```python
from build123d import *

# Parameters (mm, degrees)
SKETCH1_W      = 310
SKETCH1_H      = 180
SKETCH1_R      = 8.5
SKETCH1_R_2    = 8
EXTRUDE1_DEPTH = 6


with BuildPart() as part:
    # Sketch1 → Extrude1 (new, symmetric)
    with BuildSketch(Plane(origin=(0, 0, 0), x_dir=(1, 0, 0), z_dir=(0, 1, 0))):
        Rectangle(SKETCH1_W, SKETCH1_H)
        with Locations(Location((125, -65, 0), (0, 0, 270))):
            Circle(SKETCH1_R, mode=Mode.SUBTRACT)
        with Locations(Location((-125, -65, 0), (0, 0, 270))):
            Circle(SKETCH1_R_2, mode=Mode.SUBTRACT)
        with Locations(Location((-125, 65, 0), (0, 0, 270))):
            Circle(SKETCH1_R, mode=Mode.SUBTRACT)
        with Locations(Location((125, 65, 0), (0, 0, 270))):
            Circle(SKETCH1_R, mode=Mode.SUBTRACT)
    extrude(amount=EXTRUDE1_DEPTH, both=True)


solid = part.part
```
CAD build for the part. Positions are in the model's coordinates, mm. Round coordinates to 2 decimals unless told otherwise and drop trailing zeros. Write each loop counter-clockwise with the first axis right and the second up, starting at its lowest first coordinate (ties: lowest second). Pieces come first, ordered by that corner, then holes. Notation, with made-up numbers: (-13.5, 50) -> (30.5, 50) arc R24 ccw to (30.5, 86) -> close; hole circle Ø11 at (-10, -11.75). An arc over 180 degrees is marked (long way). Answer in a Markdown table with one row per item. Add a question column.
Item 1: Drop a flat-ended pin along its axis: pin 1 Ø15.5 at (x, z) = (-125, -65) entering from -Y. Give the stop position or say it passes through.
Item 2: Saw through at A-A, the plane x = 125. Write the cut outline in (y, z).
Item 3: Saw through at B-B, the plane z = 65. Write the cut outline in (x, y).
Item 4: Drill centre lines: line 1 (X direction, y = 1, z = -65); line 2 (X direction, y = -3, z = 65); line 3 (Z direction, x = -123, y = 0.5). Where is each one in solid material? Low to high. Write a range as from..to.
Item 5: Mould opens along X. For faces 1 (the face through (155, 0, 1)), 2 (the face through (-130.172, -0.084, -71.745)), 3 (the face through (-2, -6, -1)) say: pulls with the +X half, pulls with the -X half, needs draft (parallel to the pull), parting line crosses it, or undercut.
Findings below:
| question | item | result |
|---|---|---|
| 1 | pin 1 | passes through |
| 2 | outline | (-6, -90) -> (6, -90) -> (6, -73.5) -> (-6, -73.5) -> close; (-6, -56.5) -> (6, -56.5) -> (6, 56.5) -> (-6, 56.5) -> close; (-6, 73.5) -> (6, 73.5) -> (6, 90) -> (-6, 90) -> close |
| 3 | outline | (-155, -6) -> (-133, -6) -> (-133, 6) -> (-155, 6) -> close; (-117, -6) -> (116.5, -6) -> (116.5, 6) -> (-117, 6) -> close; (133.5, -6) -> (155, -6) -> (155, 6) -> (133.5, 6) -> close |
| 4 | line 1 | x = -155..-133.5, -116.5..116.5, 133.5..155 |
| 4 | line 2 | x = -155..-133, -117..116.5, 133.5..155 |
| 4 | line 3 | z = -90..-73.26, -56.74..57.25, 72.75..90 |
| 5 | face 1 | pulls with the +X half |
| 5 | face 2 | undercut |
| 5 | face 3 | needs draft |
